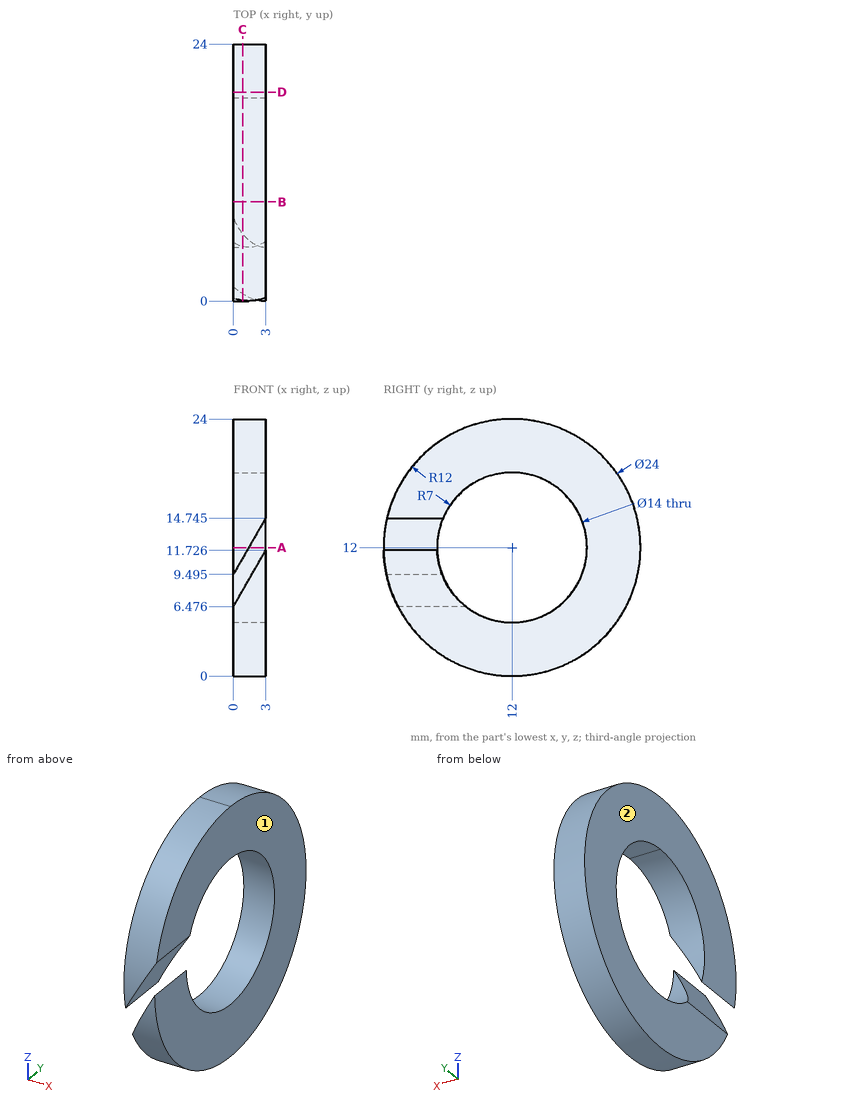
Input: dimensioned drawing with shaded views. Units: mm. Origin: part minimum x, y, z. Give positions to 0.01 mm unless a question says otherwise; leave off trailing zeros. Write each loop counter-clockwise with the first axis right and the second up, starting at its lowest first coordinate (ties: lowest second). Pieces come first, ordered by that corner, then holes. Notation, with made-up numbers: M 61,20.25 L 68,20.25 A25 cw 68,52.25 Z; hole C -14,-15 d2. An arc over 180 degrees is marked long. Write item = value, one per line. Start each with the question number.
1) Cut plane D-D on y = 19.5. Return the cut outline in (x, z).
2) Material intervals for line 1 along Y through (x, z) = (1.3, 12); line 2 along Z through (x, y) = (2.15, 9.75); line 3 along Y through (x, z) = (1.8, 12), sorted ascending. Write a range as [from, to].
3) Draft query along X for the marked faces 1 and 2. Return one class per face: +X half, -X half, draft (parallel to the pull), parting line (faces both ways), or undercut.
4) Cut plane C-C on x = 0.85. Return the cut outline in (y, z) (1 decimal), then the cut area to 3 significant figures.
5) Cut plane B-B on y = 9.25. Return the cut outline in (x, z).
6) Cut plane A-A on z = 12. Return the cut outline in (x, y).
Solved:
q1.outline = M 0,2.63 L 3,2.63 L 3,21.37 L 0,21.37 Z
q2.line_1 = [0, 5], [19, 24]
q2.line_2 = [0.21, 5.37], [18.63, 23.79]
q2.line_3 = [19, 24]
q3.face_1 = +X half
q3.face_2 = -X half
q4.outline = M 0,11 L 5.1,11 A7 cw long 6.3,8 L 0.7,8 A12 ccw long Z
q4.area = 283 mm2
q5.outline = M 0,0.32 L 3,0.32 L 3,5.56 L 0,5.56 Z; M 0,18.44 L 3,18.44 L 3,23.68 L 0,23.68 Z
q6.outline = M 0,0 L 1.43,0 L 1.43,5 L 0,5 Z; M 0,19 L 3,19 L 3,24 L 0,24 Z
